```python
from build123d import *

# Parameters (mm, degrees)
BASE_ANGLE_DEPTH           = 124
SADDLE_BOSS_DEPTH          = 50
SADDLE_SEAT_CUT_DEPTH      = 50
RELIEF_CUT_DEPTH           = 50
MOUNTING_HOLES_SKETCH_R    = 15
MOUNTING_HOLES_2X_30_DEPTH = 20


with BuildPart() as part:
    # Base Angle Profile Sketch → Base Angle (new body)
    with BuildSketch(Plane.XY):
        Polygon((0, 0), (0, 25), (50, 25), (50, 19), (8, 19), (8, 0), align=None)
    extrude(amount=BASE_ANGLE_DEPTH)

    # Saddle Boss Sketch → Saddle Boss (add)
    with BuildSketch(Plane.ZY):
        with BuildLine():
            Line((84, 65), (62, 65))
            Line((62, 65), (40, 65))
            ThreePointArc((40, 65), (44.76631206, 51.325205669), (57, 43.575714714))
            Line((57, 43.575714714), (57, 25))
            Line((57, 25), (67, 25))
            Line((67, 25), (67, 43.575714714))
            ThreePointArc((67, 43.575714714), (79.23368794, 51.325205669), (84, 65))
        make_face()
    extrude(amount=-SADDLE_BOSS_DEPTH)

    # Saddle Seat Sketch → Saddle Seat Cut (cut)
    with BuildSketch(Plane.ZY):
        with BuildLine():
            Line((48, 65), (76, 65))
            ThreePointArc((76, 65), (62, 51), (48, 65))
        make_face()
    extrude(amount=-SADDLE_SEAT_CUT_DEPTH, mode=Mode.SUBTRACT)

    # Relief Cut Sketch → Relief Cut (cut)
    with BuildSketch(Plane.ZY):
        with BuildLine():
            Line((47, 0), (77, 0))
            ThreePointArc((77, 0), (62, 15), (47, 0))
        make_face()
    extrude(amount=-RELIEF_CUT_DEPTH, mode=Mode.SUBTRACT)

    # Mounting Holes Sketch → Mounting Holes 2xØ30 (cut)
    with BuildSketch(Plane.XZ.offset(-19)):
        with Locations(Location((25, 94, 0), (0, 0, 270))):
            Circle(MOUNTING_HOLES_SKETCH_R)
        with Locations(Location((25, 30, 0), (0, 0, 270))):
            Circle(MOUNTING_HOLES_SKETCH_R)
    extrude(amount=-MOUNTING_HOLES_2X_30_DEPTH, mode=Mode.SUBTRACT)


solid = part.part
```
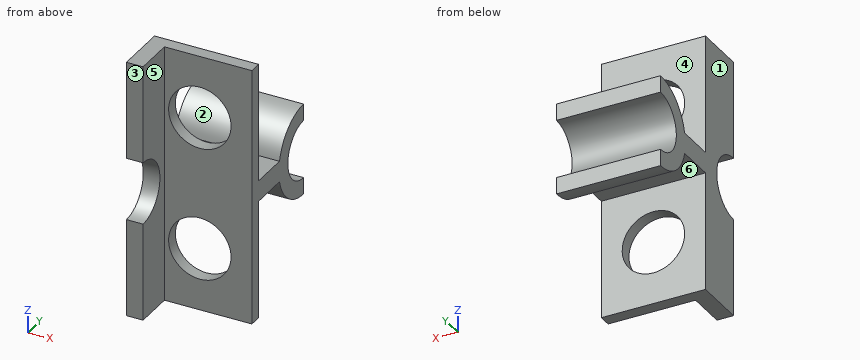
Check sheet for the modelled part. Datum: model origin and axes. Units: mm. Face numbers are marked on the shaded views. A direction names the side the tool comes from. Give positions to 0.01 mm unless a question says otherwise; leave off trailing zeros. Order: outer loops, then holes, each group sorted by start corner. A loop starts at its lowest first (then second) coordinate and runs counter-clockwise, first axis right, second up. Notation, with made-up numbers: M 42,-30 L 85,-30 A12 ccw 85,-15 Z; hole C -10,38.25 d3. An arc over 180 degrees is marked long. Answer in a Markdown table with one row per item. Add a question column.
Q1. Release check for a two-part mould opening along Y. For the marked faces 1, 2 and 3 record: released by +Y, released by -Y, zero draft, split by the parting line, or undercut.
Q2. Gauge pin test, flat ends, axial feed: pin 1 Ø4 at (x, z) = (16, 62.5) entering from +Y (3 decimals); pin 2 Ø9.5 at (x, y) = (21.5, 31) entering from +Z; pin 3 Ø1 at (x, z) = (33.5, 75) entering from -Y. Record the tip position at first contact, or that the pin passes through.
Q3. Sectioned sample at D-D, the plane x = 41.5. Record the boundary of the cut face in (y, z).
Q4. Thickness scan on L1, parallel to X at y = 21.6, z = 94; L2, parallel to Z at x = 17, y = 24; L3, parallel to Z at x = 27.5, y = 24. Record the ranges inside material, lowest first.
Q5. Sectioned sample at A-A, the plane z = 94. Record the boundary of the cut face in (x, y), and give its area (3 significant figures).
Q6. Sectioned sample at C-C, the plane x = 34.5. Record the boundary of the cut face in (y, z), and give its area (3 significant figures).
Q7. Sectioned sample at B-B, the plane y = 60.5. Record the boundary of the cut face in (x, z).
Q8. Access from +Z, -Z, +X, -X, +Y, -Y to the whole of each face (thin tool, end or side, straight path). Record for the marked faces 4, 5 and 6.
Verdict:
| question | item | result |
|---|---|---|
| 1 | face 1 | zero draft |
| 1 | face 2 | undercut |
| 1 | face 3 | released by -Y |
| 2 | pin 1 | y = 51.225 |
| 2 | pin 2 | z = 67 |
| 2 | pin 3 | y = 19 |
| 3 | outline | M 19,0 L 25,0 L 25,57 L 43.58,57 A22 ccw 65,40 L 65,48 A14 cw 65,76 L 65,84 A22 ccw 43.58,67 L 25,67 L 25,124 L 19,124 Z |
| 4 | L1 | 0 to 10, 40 to 50 |
| 4 | L2 | 0 to 17.31, 42.69 to 81.31, 106.69 to 124 |
| 4 | L3 | 0 to 15.21, 44.79 to 79.21, 108.79 to 124 |
| 5 | outline | M 0,0 L 8,0 L 8,19 L 10,19 L 10,25 L 0,25 Z; M 40,19 L 50,19 L 50,25 L 40,25 Z |
| 5 | area | 272 mm² |
| 6 | outline | M 19,0 L 25,0 L 25,18.39 L 19,18.39 Z; M 19,41.61 L 25,41.61 L 25,57 L 43.58,57 A22 ccw 65,40 L 65,48 A14 cw 65,76 L 65,84 A22 ccw 43.58,67 L 25,67 L 25,82.39 L 19,82.39 Z; M 19,105.61 L 25,105.61 L 25,124 L 19,124 Z |
| 6 | area | 1,100 mm² |
| 7 | outline | M 0,40.47 L 50,40.47 L 50,48.74 L 0,48.74 Z; M 0,75.26 L 50,75.26 L 50,83.53 L 0,83.53 Z |
| 8 | face 4 | +Z, +X, -X |
| 8 | face 5 | +Z, -Z, +X, -Y |
| 8 | face 6 | -Z, +X, -X |
